Read the model definition and answer for the solid it produces. Units are mm, in the model's axes. Face numbers are marked on the shaded views. A direction names the side the tool comes from. Round coordinates to 2 decimals unless told otherwise and drop trailing zeros. Write each loop counter-clockwise with the first axis right and the second up, starting at its lowest first coordinate (ties: lowest second). Pieces come first, ordered by that corner, then holes. Notation, with made-up numbers: (4.5, 12) - (44.5, 12) arc R26 ccw to (44.5, 33) - close; hole circle Ø5 at (-9, 11). An arc over 180 degrees is marked (long way). Use one line per item in the form item = value. Start each with the question number.
1) The part is cut by section A-A, the plane x = 15. Give the vertices of the cut face in (y, z), plus the area to 3 significant figures.
2) Consider line 1 along X through (y, z) = (-14.25, 50); line 2 along Z through (x, y) = (17, -15.25); line 3 along Y through (x, z) = (22.5, 28). Determine where each line is inside the solid, lowest interval first. Write a range as from..to.
3) The part is cut by section B-B, the plane z = 26.5. Give the vertices of the cut face in (x, y), plus the area to 3 significant figures.
4) Each of these flat-tipped pins is pushed along its axis until it touches: pin 1 (3 mm diameter, centred on x = 19.5, z = 23.5, fed in from +Y); pin 2 (5 mm diameter, centred on x = 15, z = 10, fed in from +Y). Where does it stop, or does it pass through?
5) For the marked faces 1 and 2, determine the directions among +Z, -Z, +X, -X, +Y, -Y from which every point of the face is accessible in a straight line to the end or side of a thin tool.
6) The part is cut by section D-D, the plane x = 29. Give the vertices of the cut face in (y, z), plus the area to 3 significant figures.
7) For a pull along X with two mould halves and no side action, classify the marked faces 3, 4 and 5 as released by +X, released by -X, zero draft, split by the parting line, or undercut.
8) The part is cut by section C-C, the plane y = -13.25. Give the vertices of the cut face in (x, z).
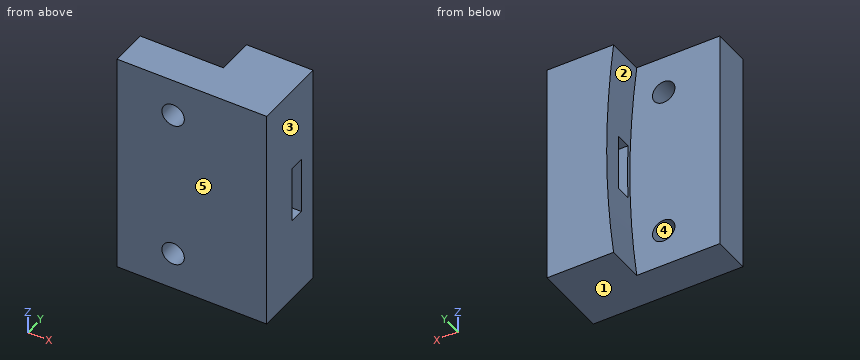
from build123d import *

# Parameters (mm, degrees)
SKETCH1_W           = 40
SKETCH1_H           = 20
BOSS_EXTRUDE1_DEPTH = 60
CUT_EXTRUDE1_DEPTH  = 10
SKETCH3_R           = 3
CUT_EXTRUDE2_DEPTH  = 10
SKETCH4_W           = 15
SKETCH4_H           = 4
CUT_EXTRUDE3_DEPTH  = 49


with BuildPart() as part:
    # Sketch1 → Boss-Extrude1 (new body)
    with BuildSketch(Plane.XY):
        with Locations((20, -10)):
            Rectangle(SKETCH1_W, SKETCH1_H)
    extrude(amount=BOSS_EXTRUDE1_DEPTH)

    # Sketch2 → Cut-Extrude1 (cut)
    with BuildSketch(Plane(origin=(0, 0, 0), x_dir=(1, 0, 0), z_dir=(0, 1, 0))):
        with BuildLine():
            Line((22.2, 0), (0, 0))
            Line((0, 0), (0, -60))
            Line((0, -60), (22.2, -60))
            ThreePointArc((22.2, -60), (24.043671684, -30), (22.2, 0))
        make_face()
    extrude(amount=-CUT_EXTRUDE1_DEPTH, mode=Mode.SUBTRACT)

    # Sketch3 → Cut-Extrude2 (cut)
    with BuildSketch(Plane(origin=(0, -10, 0), x_dir=(1, 0, 0), z_dir=(0, 1, 0))):
        with Locations(Location((15, -10, 0), (0, 0, 270))):
            Circle(SKETCH3_R)
        with Locations(Location((15, -50, 0), (0, 0, 270))):
            Circle(SKETCH3_R)
    extrude(amount=-CUT_EXTRUDE2_DEPTH, mode=Mode.SUBTRACT)

    # Sketch4 → Cut-Extrude3 (cut)
    with BuildSketch(Plane(origin=(40, 0, 0), x_dir=(0, 0, -1), z_dir=(1, 0, 0))):
        with Locations((-30, -7)):
            Rectangle(SKETCH4_W, SKETCH4_H)
    extrude(amount=-CUT_EXTRUDE3_DEPTH, mode=Mode.SUBTRACT)


solid = part.part
Geometry results:
q1.outline = (-20, 0) - (-10, 0) - (-10, 7) - (-20, 7) - close; (-20, 13) - (-10, 13) - (-10, 47) - (-20, 47) - close; (-20, 53) - (-10, 53) - (-10, 60) - (-20, 60) - close
q1.area = 480 mm2
q2.line_1 = 0..12, 18..40
q2.line_2 = 0..7.76, 12.24..47.76, 52.24..60
q2.line_3 = -20..-10
q3.outline = (0, -20) - (40, -20) - (40, -9) - (24.02, -9) - (24.02, -10) - (0, -10) - close; (24.02, -5) - (40, -5) - (40, 0) - (24.02, 0) - close
q3.area = 496 mm2
q4.pin_1 = -10
q4.pin_2 = through
q5.face_1 = -Z, +X, -X, +Y, -Y
q5.face_2 = -X, +Y
q6.outline = (-20, 0) - (0, 0) - (0, 60) - (-20, 60) - close; hole (-9, 22.5) - (-5, 22.5) - (-5, 37.5) - (-9, 37.5) - close
q6.area = 1,140 mm2
q7.face_3 = released by +X
q7.face_4 = undercut
q7.face_5 = zero draft
q8.outline = (0, 0) - (40, 0) - (40, 60) - (0, 60) - close; hole circle Ø6 at (15, 10); hole circle Ø6 at (15, 50)
